Here's how the part is built. I have some questions about the finished solid (model axes, mm). A direction names the side the tool comes from. Round coordinates to 2 decimals unless told otherwise and drop trailing zeros. Loops run counter-clockwise (first coordinate to the right, second up) from the corner with the lowest first, then second, coordinate; pieces in that order, holes last. Notation, with made-up numbers: M 14,21.25 L 56,21.25 A35 ccw 56,60.25 Z; hole C -2,58.25 d6. An arc over 180 degrees is marked long. Answer as a JSON object with one key per item and string values.
from build123d import *

# Parameters (mm, degrees)
BASE_PLATE_SKETCH_W           = 150
BASE_PLATE_SKETCH_H           = 100
BASE_PLATE_150X100X25_DEPTH   = 25
UPRIGHT_PLATE_SKETCH_W        = 25
UPRIGHT_PLATE_SKETCH_H        = 100
UPRIGHT_PLATE_DEPTH           = 65
ANGLED_BOSS_REACH             = 179.236
BOSS_SLOT_REACH               = 149.733
BOSS_BORE_REACH               = 179.236
BOSS_BORE_SKETCH_R            = 15
BASE_PLATE_HOLES_REACH        = 129.377
BASE_PLATE_HOLES_SKETCH_R     = 10
UPRIGHT_PLATE_HOLES_REACH     = 183.934
UPRIGHT_PLATE_HOLES_SKETCH_R  = 10
UPRIGHT_CORNER_FILLET_R25_A_R = 25
UPRIGHT_CORNER_FILLET_R25_B_R = 25
BASE_CORNER_FILLET_R25_A_R    = 25
BASE_CORNER_FILLET_R25_B_R    = 25


with BuildPart() as part:
    # Base Plate Sketch → Base Plate 150x100x25 (new body)
    with BuildSketch(Plane.XY):
        Rectangle(BASE_PLATE_SKETCH_W, BASE_PLATE_SKETCH_H)
    extrude(amount=BASE_PLATE_150X100X25_DEPTH)

    # Upright Plate Sketch → Upright Plate (add)
    with BuildSketch(Plane.XY.offset(25)):
        with Locations((-62.5, 0)):
            Rectangle(UPRIGHT_PLATE_SKETCH_W, UPRIGHT_PLATE_SKETCH_H)
    extrude(amount=UPRIGHT_PLATE_DEPTH)

    # Angled Boss Sketch → Angled Boss (add, up to next)
    with BuildSketch(Plane(origin=(-37.5, 0, -37.5), x_dir=(0.7071067811865512, 0, -0.7071067811865439), z_dir=(0.7071067811865439, 0, 0.7071067811865512)), mode=Mode.PRIVATE) as angled_boss_sk1:
        with BuildLine():
            Line((-53.033008589, 40), (1.966991411, 40))
            ThreePointArc((1.966991411, 40), (41.966991411, 0), (1.966991411, -40))
            Line((1.966991411, -40), (-53.033008589, -40))
            Line((-53.033008589, -40), (-53.033008589, 40))
        make_face()
    angled_boss_tool1 = extrude(angled_boss_sk1.sketch, amount=ANGLED_BOSS_REACH, mode=Mode.PRIVATE) - part.part
    add(angled_boss_tool1.solids().sort_by_distance((-44.121254, 0, -30.878746))[0])

    # Boss Slot Sketch → Boss Slot (cut, up to next)
    with BuildSketch(Plane(origin=(0, 40, 0), x_dir=(1, 0, 0), z_dir=(0, 1, 0)), mode=Mode.PRIVATE) as boss_slot_sk1:
        Polygon((-57.32233047, 17.67766953), (-46.715728753, 7.071067812), (-36.109127035, 17.67766953), (-46.715728753, 28.284271247), align=None)
    boss_slot_tool1 = extrude(boss_slot_sk1.sketch, amount=-BOSS_SLOT_REACH, mode=Mode.PRIVATE) & part.part
    add(boss_slot_tool1.solids().sort_by_distance((-46.715729, 40, -17.67767))[0], mode=Mode.SUBTRACT)

    # Boss Bore: up to this plane
    boss_bore_end = Plane(origin=(0, 0, 25), z_dir=(0, 0, -1))
    # Boss Bore Sketch → Boss Bore (cut, up to the surface)
    with BuildSketch(Plane(origin=(-37.5, 0, -37.5), x_dir=(-0.7071067811865511, 0, 0.707106781186544), z_dir=(-0.707106781186544, 0, -0.7071067811865511)), mode=Mode.PRIVATE) as boss_bore_sk1:
        with Locations((-6.966991411, 0)):
            Circle(BOSS_BORE_SKETCH_R)
    boss_bore_tool1 = split(extrude(boss_bore_sk1.sketch, amount=-BOSS_BORE_REACH, mode=Mode.PRIVATE), bisect_by=boss_bore_end, keep=Keep.BOTH, mode=Mode.PRIVATE)
    add(boss_bore_tool1.solids().sort_by_distance((-32.573593, 0, -42.426407))[0], mode=Mode.SUBTRACT)

    # Base Plate Holes Sketch → Base Plate Holes (cut, up to next)
    with BuildSketch(Plane(origin=(0, 0, 0), x_dir=(-1, 0, 0), z_dir=(0, 0, -1)), mode=Mode.PRIVATE) as base_plate_holes_sk1:
        with Locations((-60, 30)):
            Circle(BASE_PLATE_HOLES_SKETCH_R)
    base_plate_holes_tool1 = extrude(base_plate_holes_sk1.sketch, amount=-BASE_PLATE_HOLES_REACH, mode=Mode.PRIVATE) & part.part
    # Base Plate Holes Sketch → Base Plate Holes (cut, up to next)
    with BuildSketch(Plane(origin=(0, 0, 0), x_dir=(-1, 0, 0), z_dir=(0, 0, -1)), mode=Mode.PRIVATE) as base_plate_holes_sk2:
        with Locations((-60, -30)):
            Circle(BASE_PLATE_HOLES_SKETCH_R)
    base_plate_holes_tool2 = extrude(base_plate_holes_sk2.sketch, amount=-BASE_PLATE_HOLES_REACH, mode=Mode.PRIVATE) & part.part
    add(base_plate_holes_tool1.solids().sort_by_distance((60, 30, 0))[0], mode=Mode.SUBTRACT)
    add(base_plate_holes_tool2.solids().sort_by_distance((60, -30, 0))[0], mode=Mode.SUBTRACT)

    # Upright Plate Holes Sketch → Upright Plate Holes (cut, up to next)
    with BuildSketch(Plane.ZY.offset(75), mode=Mode.PRIVATE) as upright_plate_holes_sk1:
        with Locations((70, 30)):
            Circle(UPRIGHT_PLATE_HOLES_SKETCH_R)
    upright_plate_holes_tool1 = extrude(upright_plate_holes_sk1.sketch, amount=-UPRIGHT_PLATE_HOLES_REACH, mode=Mode.PRIVATE) & part.part
    # Upright Plate Holes Sketch → Upright Plate Holes (cut, up to next)
    with BuildSketch(Plane.ZY.offset(75), mode=Mode.PRIVATE) as upright_plate_holes_sk2:
        with Locations((70, -30)):
            Circle(UPRIGHT_PLATE_HOLES_SKETCH_R)
    upright_plate_holes_tool2 = extrude(upright_plate_holes_sk2.sketch, amount=-UPRIGHT_PLATE_HOLES_REACH, mode=Mode.PRIVATE) & part.part
    add(upright_plate_holes_tool1.solids().sort_by_distance((-75, 30, 70))[0], mode=Mode.SUBTRACT)
    add(upright_plate_holes_tool2.solids().sort_by_distance((-75, -30, 70))[0], mode=Mode.SUBTRACT)

    # Upright Corner Fillet R25 A
    upright_corner_fillet_r25_a_edges = [part.edges().sort_by_distance(p)[0] for p in [
        (-62.5, 50, 90),
    ]]
    fillet(upright_corner_fillet_r25_a_edges, radius=UPRIGHT_CORNER_FILLET_R25_A_R)

    # Upright Corner Fillet R25 B
    upright_corner_fillet_r25_b_edges = [part.edges().sort_by_distance(p)[0] for p in [
        (-62.5, -50, 90),
    ]]
    fillet(upright_corner_fillet_r25_b_edges, radius=UPRIGHT_CORNER_FILLET_R25_B_R)

    # Base Corner Fillet R25 A
    base_corner_fillet_r25_a_edges = [part.edges().sort_by_distance(p)[0] for p in [
        (75, -50, 12.5),
    ]]
    fillet(base_corner_fillet_r25_a_edges, radius=BASE_CORNER_FILLET_R25_A_R)

    # Base Corner Fillet R25 B
    base_corner_fillet_r25_b_edges = [part.edges().sort_by_distance(p)[0] for p in [
        (75, 50, 12.5),
    ]]
    fillet(base_corner_fillet_r25_b_edges, radius=BASE_CORNER_FILLET_R25_B_R)


solid = part.part
Item 1: I'm going to push flat-ended pins straight in: pin 1 Ø18 at (y, z) = (-30, 70) entering from +X; pin 2 Ø19.5 at (y, z) = (-2, 59) entering from +X; pin 3 Ø1 at (x, y) = (-60, -22.5) entering from -Z; pin 4 Ø6 at (y, z) = (9, -31) entering from -X. Where does each tip first touch, or does it pass through?
Resolved:
{"pin 1": "through", "pin 2": "x = -50", "pin 3": "z = -15.5", "pin 4": "x = -46.72"}
Item 2: I want a section at B-B, the plane y = -30. Please give me the cut outline in (x, z).
Resolved:
{"outline": "M -75,0 L -57.32,-17.68 L -46.72,-7.07 L -36.11,-17.68 L -46.72,-28.28 L -17.4,-57.6 L 40.2,0 L 50,0 L 50,25 L -50,25 L -50,60 L -75,60 Z; M -75,80 L -50,80 L -50,89.49 L -75,89.49 Z; M 70,0 L 74.49,0 L 74.49,25 L 70,25 Z"}
Item 3: I want a section at D-D, the plane z = 44.5. Please give me the cut outline in (x, y), then the cut area to 3 significant figures.
Resolved:
{"outline": "M -75,-50 L -50,-50 L -50,50 L -75,50 Z", "area": "2,500 mm²"}
Item 4: If we mould it in two halves opening along Z, with no side actions, what happens to faces 6 (the face through (-63, 24, 62)), 7 (the face through (-41.487, 0.56, -12.3)), 8 (the face through (-62.325, 42.482, 82.871)), 9 (the face through (-27, 50, 18))? For each: pulls with the +Z half, pulls with the -Z half, needs draft (parallel to the pull), parting line crosses it, or undercut.
Resolved:
{"face 6": "undercut", "face 7": "undercut", "face 8": "pulls with the +Z half", "face 9": "needs draft"}
Item 5: On a 3-axis mill with a long thin cutter (end or side, diameter ignored), from which of +Z, -Z, +X, -X, +Y, -Y can I reach the whole of each face in a straight line? I mean faces 1 (the face through (-75, -1, 44)), 2 (the face through (-33, 40, -12)), 3 (the face through (-2, 1, 25)), 4 (the face through (27, 37, 0)), 5 (the face through (-36, -40, -9)). Say none if no direction works.
Resolved:
{"face 1": "+Z, -Z, -X, +Y, -Y", "face 2": "-Z, +X, -X, +Y", "face 3": "+Z, +X, +Y, -Y", "face 4": "-Z, +X", "face 5": "-Z, +X, -X, -Y"}
Item 6: I want a section at A-A, the plane z = 70. Please give me the cut outline in (x, y).
Resolved:
{"outline": "M -75,-49.49 L -50,-49.49 L -50,-40 L -75,-40 Z; M -75,-20 L -50,-20 L -50,20 L -75,20 Z; M -75,40 L -50,40 L -50,49.49 L -75,49.49 Z"}
Item 7: Please list where these lines run through material, in increasing order: probe 1 along Y at (x, z) = (60, 18.5); probe 2 along Y at (x, z) = (-61, 70); probe 3 along Z at (x, y) = (54, -17). Write a range as from..to.
Resolved:
{"probe 1": "-47.91..-40, -20..20, 40..47.91", "probe 2": "-49.49..-40, -20..20, 40..49.49", "probe 3": "0..25"}
Item 8: I want a section at C-C, the plane y = -18. Please give me the cut outline in (x, z).
Resolved:
{"outline": "M -75,0 L -57.32,-17.68 L -46.72,-7.07 L -36.11,-17.68 L -46.72,-28.28 L -10.85,-64.15 L 53.3,0 L 75,0 L 75,25 L -50,25 L -50,90 L -75,90 Z"}
